CAD build for the part. Positions are in the model's coordinates, mm. Face numbers are marked on the shaded views. Coordinates: 2 decimals unless noted, no trailing zeros. Loops run counter-clockwise (first coordinate to the right, second up) from the corner with the lowest first, then second, coordinate; pieces in that order, holes last. Notation, with made-up numbers: (-29, -19) -> (8, -19) arc R15 cw to (8, -11) -> close; hole circle Ø6 at (12.25, 70.5). An arc over 180 degrees is marked (long way). Write each question's results on one line, items separated by ' | '.
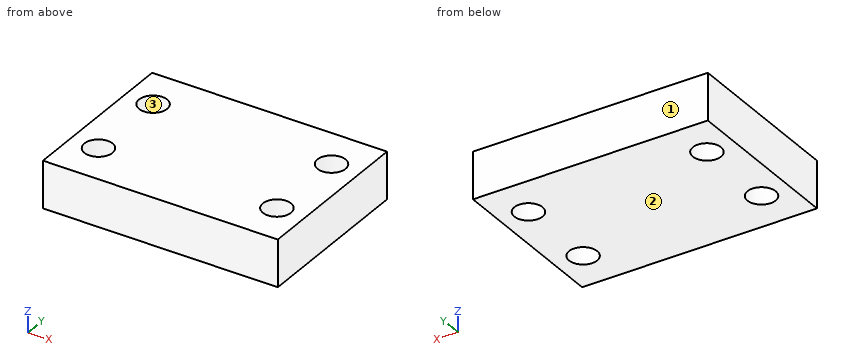
from build123d import *

# Parameters (mm, degrees)
SKETCH1_W           = 25
SKETCH1_H           = 18
SKETCH1_R           = 1.5
BOSS_EXTRUDE1_DEPTH = 5


with BuildPart() as part:
    # Sketch1 → Boss-Extrude1 (new body)
    with BuildSketch(Plane.XY):
        Rectangle(SKETCH1_W, SKETCH1_H)
        with Locations((-9.5, 4.5)):
            Circle(SKETCH1_R, mode=Mode.SUBTRACT)
        with Locations((9.5, 4.5)):
            Circle(SKETCH1_R, mode=Mode.SUBTRACT)
        with Locations((9.5, -4.5)):
            Circle(SKETCH1_R, mode=Mode.SUBTRACT)
        with Locations((-9.5, -4.5)):
            Circle(SKETCH1_R, mode=Mode.SUBTRACT)
    extrude(amount=BOSS_EXTRUDE1_DEPTH)


solid = part.part
1) Pin check, flat tips, straight feed: pin 1 (5 mm diameter, centred on x = -1, y = 0.5, fed in from -Z); pin 2 (2.5 mm diameter, centred on x = 9.5, y = 4.5, fed in from -Z). Stop position of each tip, or through.
Outcome:
pin 1: stops at z = 0 | pin 2: passes through
2) Slice it at C-C (y = 4.5). Write the cut outline in (x, z), then the cut area to 3 significant figures.
Outcome:
outline: (-12.5, 0) -> (-11, 0) -> (-11, 5) -> (-12.5, 5) -> close; (-8, 0) -> (8, 0) -> (8, 5) -> (-8, 5) -> close; (11, 0) -> (12.5, 0) -> (12.5, 5) -> (11, 5) -> close | area: 95.0 mm^2
3) Two-plate mould, pull along Y, no slides. Class the marked faces 1, 2 and 3: pulls with the +Y half, pulls with the -Y half, needs draft (parallel to the pull), parting line crosses it, or undercut.
Outcome:
face 1: pulls with the +Y half | face 2: needs draft | face 3: undercut
4) Drill centre lines: L1, parallel to Y at x = -9.5, z = 3.35; L2, parallel to Y at x = 10.75, z = 0.75; L3, parallel to X at y = 4, z = 3.3. Where is each one in solid material? Low to high. Write a range as from..to.
Outcome:
L1: y = -9..-6, -3..3, 6..9 | L2: y = -9..-5.33, -3.67..3.67, 5.33..9 | L3: x = -12.5..-10.91, -8.09..8.09, 10.91..12.5
5) Slice it at B-B (x = 9.5). Write the cut outline in (y, z), then the cut area to 3 significant figures.
Outcome:
outline: (-9, 0) -> (-6, 0) -> (-6, 5) -> (-9, 5) -> close; (-3, 0) -> (3, 0) -> (3, 5) -> (-3, 5) -> close; (6, 0) -> (9, 0) -> (9, 5) -> (6, 5) -> close | area: 60.0 mm^2
6) Slice it at A-A (z = 4.7). Write the cut outline in (x, y), then the cut area to 3 significant figures.
Outcome:
outline: (-12.5, -9) -> (12.5, -9) -> (12.5, 9) -> (-12.5, 9) -> close; hole circle Ø3 at (-9.5, -4.5); hole circle Ø3 at (-9.5, 4.5); hole circle Ø3 at (9.5, -4.5); hole circle Ø3 at (9.5, 4.5) | area: 422 mm^2
